```python
from build123d import *

# Parameters (mm, degrees)
EXTRUDE_1_DEPTH    = 7
HOLE_WIZARD_M3_1_D = 2.5


with BuildPart() as part:
    # 草图1 → 凸台-拉伸1 (new body)
    with BuildSketch(Plane(origin=(0, 0, 0), x_dir=(0, 0, -1), z_dir=(1, 0, 0))):
        Polygon((2.655811238, 0), (1.327905619, 2.3), (-1.327905619, 2.3), (-2.655811238, 0), (-1.327905619, -2.3), (1.327905619, -2.3), align=None)
    extrude(amount=EXTRUDE_1_DEPTH)

    # M3 螺纹孔1 (through all)
    with Locations(Plane(origin=(7, 0, 0), x_dir=(0, 0, -1), z_dir=(1, 0, 0))):
        with Locations((0, 0)):
            Hole(HOLE_WIZARD_M3_1_D / 2)


solid = part.part
```
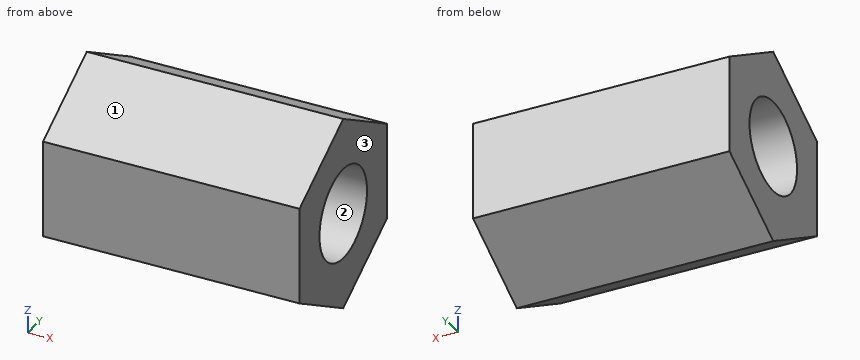
CAD build for the part. Positions are in the model's coordinates, mm. Face numbers are marked on the shaded views. Coordinates: 2 decimals unless noted, no trailing zeros. Write each loop counter-clockwise with the first axis right and the second up, starting at its lowest first coordinate (ties: lowest second). Pieces come first, ordered by that corner, then holes. Notation, with made-up numbers: (29.25, 15) -> (82.25, 15) arc R29 cw to (82.25, 52) -> close; hole circle Ø1 at (42, -25.75). An arc over 180 degrees is marked (long way). Use CSV: the item, a comma, the result in double quotes. Start each with the question number.
Item 1: Band-saw the part on C-C, the plane x = 1.25. Write the cut outline in (y, z).
Item 2: Two-plate mould, pull along Z, no slides. Class the marked faces 1, 2 and 3: +Z half, -Z half, draft (parallel to the pull), parting line (faces both ways), or undercut.
Item 3: Band-saw the part on D-D, the plane z = 2.2. Write the cut outline in (x, y), plus the area to 3 significant figures.
Item 4: Wall check: probe 1 along Y at (x, z) = (5.75, 0); probe 2 along Z at (x, y) = (5.25, 1); probe 3 along Y at (x, z) = (1.5, 1.85). Give the ranges that are in metal, low to high.
Item 5: Band-saw the part on B-B, the plane y = 1. Write the cut outline in (x, z).
Item 6: Drop a flat-ended pin along its axis: P1, Ø1, axis at x = 4, y = 1, coming from the +Z side. Give the stop position or say it passes through.
Item 7: Band-saw the part on A-A, the plane z = 0. Write the cut outline in (x, y).
Response values:
1,outline,"(-2.3, -1.33) -> (0, -2.66) -> (2.3, -1.33) -> (2.3, 1.33) -> (0, 2.66) -> (-2.3, 1.33) -> close; hole circle Ø2.5 at (0, 0)"
2,face 1,"+Z half"
2,face 2,"undercut"
2,face 3,"draft"
3,outline,"(0, -0.79) -> (7, -0.79) -> (7, 0.79) -> (0, 0.79) -> close"
3,area,"11.1 mm2"
4,probe 1,"y = -2.3 to -1.25, 1.25 to 2.3"
4,probe 2,"z = -2.08 to -0.75, 0.75 to 2.08"
4,probe 3,"y = -1.4 to 1.4"
5,outline,"(0, -2.08) -> (7, -2.08) -> (7, -0.75) -> (0, -0.75) -> close; (0, 0.75) -> (7, 0.75) -> (7, 2.08) -> (0, 2.08) -> close"
6,P1,"stops at z = 2.37"
7,outline,"(0, -2.3) -> (7, -2.3) -> (7, -1.25) -> (0, -1.25) -> close; (0, 1.25) -> (7, 1.25) -> (7, 2.3) -> (0, 2.3) -> close"
